The listing builds one solid part. Answer for the finished solid, in the listing's coordinates (mm). A direction names the side the tool comes from. Round coordinates to 2 decimals unless told otherwise and drop trailing zeros. Loops run counter-clockwise (first coordinate to the right, second up) from the corner with the lowest first, then second, coordinate; pieces in that order, holes last. Notation, with made-up numbers: (-15, 47) -> (3, 47) arc R25 ccw to (3, 77) -> close; hole circle Ø7 at (-3, -37). An arc over 180 degrees is marked (long way). Use a Markdown table: item, result. Add a question column.
Q1. Section C-C on y = 77 is taken. Give the vertices of the cut face in (x, z).
Q2. Section A-A on z = 0 is taken. Give the vertices of the cut face in (x, y), then the cut area to 3 significant figures.
Q3. Which of the six approach directions +Z, -Z, +X, -X, +Y, -Y give full straight-line access (tool end or side, diameter ignored) to faces 4 (the cylindrical face through (91.048, 28.025, -0.879)), 5 (the flat face through (69, 107.791, -15)), 6 (the cylindrical face through (52.039, 95.988, -5.992))?
Q4. For a pull along Z with two mould halves and no side action, classify faces 1 (the cylindrical face through (47.22, 28.74, -7.51)), 2 (the flat face through (82, -25.489, -17)), 3 (the cylindrical face through (86, 94.1, -0.7)) as released by +Z, released by -Z, zero draft, split by the parting line, or undercut.
Q5. Consider line 1 (X direction, y = 46, z = -1); line 2 (X direction, y = 10, z = 0); line 3 (Y direction, x = 72.5, z = 21). Determine where each line is inside the solid, lowest interval first.
Q6. Given pin 1 Ø12 at (x, y) = (79, 68.5) entering from -Z; pin 2 Ø20 at (x, z) = (77.5, -7.5) entering from -Y; pin 3 Ø24 at (x, z) = (71.07, 0) entering from +Y; pin 4 Ø12 at (x, y) = (70.5, 38.5) entering from +Z, each flat-ended and moving along its own axis, determine where each tip first touches the part or whether it passes through.
Q7. Section B-B on x = 77 is taken. Give the vertices of the cut face in (y, z).
from build123d import *


with BuildPart() as part:
    # Sketch2 → Revolve1 (revolve)
    with BuildSketch(Plane.XY):
        Polygon((51.067350004, -25.488807327), (51.067350004, 80.061192673), (56.117350004, 80.061192673), (56.117350004, 107.791192673), (51.117350004, 107.791192673), (51.117350004, 97.791192673), (51.117350004, 84.511192673), (46.067350004, 84.511192673), (46.067350004, -25.488807327), align=None)
    revolve(axis=Axis((71.067350004, 101.177656429, 0), (0, -1, 0)))


solid = part.part
Checked values:
| question | item | result |
|---|---|---|
| 1 | outline | circle Ø50 at (71.07, 0); hole circle Ø40 at (71.07, 0) |
| 2 | outline | (46.07, -25.49) -> (51.07, -25.49) -> (51.07, 80.06) -> (56.12, 80.06) -> (56.12, 107.79) -> (51.12, 107.79) -> (51.12, 84.51) -> (46.07, 84.51) -> close; (86.02, 80.06) -> (91.07, 80.06) -> (91.07, -25.49) -> (96.07, -25.49) -> (96.07, 84.51) -> (91.02, 84.51) -> (91.02, 107.79) -> (86.02, 107.79) -> close |
| 2 | area | 1,380 mm2 |
| 3 | face 4 | -Y |
| 3 | face 5 | +Z, -Z, +X, -X, +Y |
| 3 | face 6 | +Y |
| 4 | face 1 | split by the parting line |
| 4 | face 2 | zero draft |
| 4 | face 3 | undercut |
| 5 | line 1 | x = 46.09 to 51.09, 91.04 to 96.05 |
| 5 | line 2 | x = 46.07 to 51.07, 91.07 to 96.07 |
| 5 | line 3 | y = -25.49 to 84.51 |
| 6 | pin 1 | stops at z = -24.93 |
| 6 | pin 2 | stops at y = 80.06 |
| 6 | pin 3 | passes through |
| 6 | pin 4 | stops at z = 25 |
| 7 | outline | (-25.49, -24.29) -> (84.51, -24.29) -> (84.51, -19.05) -> (107.79, -19.05) -> (107.79, -13.72) -> (80.06, -13.72) -> (80.06, -19.1) -> (-25.49, -19.1) -> close; (-25.49, 19.1) -> (80.06, 19.1) -> (80.06, 13.72) -> (107.79, 13.72) -> (107.79, 19.05) -> (84.51, 19.05) -> (84.51, 24.29) -> (-25.49, 24.29) -> close |
